```python
from build123d import *

# Parameters (mm, degrees)
SKETCH_1_W                = 80
SKETCH_1_H                = 80
EXTRUDE_1_DEPTH           = 80
HOLE_WIZARD_1_D           = 11
HOLE_WIZARD_1_CBORE_D     = 18
HOLE_WIZARD_1_CBORE_DEPTH = 50
CUT_EXTRUDE_1_DEPTH       = 121


with BuildPart() as part:
    # 草图1 → 凸台-拉伸1 (new body)
    with BuildSketch(Plane(origin=(0, 0, 0), x_dir=(0, 0, -1), z_dir=(1, 0, 0))):
        Rectangle(SKETCH_1_W, SKETCH_1_H)
    extrude(amount=EXTRUDE_1_DEPTH)

    # 打孔尺寸(%根据)内六角圆柱头螺钉的类型1 (through all)
    with Locations(Plane(origin=(80, 0, 0), x_dir=(0, 0, -1), z_dir=(1, 0, 0))):
        with Locations((-25, 0), (25, 0)):
            CounterBoreHole(HOLE_WIZARD_1_D / 2, HOLE_WIZARD_1_CBORE_D / 2, HOLE_WIZARD_1_CBORE_DEPTH)

    # 草图2 → 切除-拉伸1 (cut, through all)
    with BuildSketch(Plane.XY.offset(40)):
        Polygon((20, -40), (80, 20), (80, -40), align=None)
    extrude(amount=-CUT_EXTRUDE_1_DEPTH, mode=Mode.SUBTRACT)


solid = part.part
```
Can you work these out from the model? Positions are in its coordinate system, mm. A direction names the side the tool comes from. Coordinates: 2 decimals unless noted, no trailing zeros. Loops run counter-clockwise (first coordinate to the right, second up) from the corner with the lowest first, then second, coordinate; pieces in that order, holes last.
Item 1: I'm going to push flat-ended pins straight in: pin 1 (9 mm diameter, centred on y = -3, z = 27, fed in from +X); pin 2 (12 mm diameter, centred on x = 56, y = -14.5, fed in from -Z); pin 3 (6 mm diameter, centred on y = -19, z = 17.5, fed in from +X); pin 4 (1.5 mm diameter, centred on x = 35.5, z = -10, fed in from -Y). Where does each tip first touch, or does it pass through?
Answers below:
pin 1: stops at x = 30
pin 2: passes through
pin 3: stops at x = 44
pin 4: stops at y = -25.25
Item 2: Suppose I cut it at D-D (x = 54). Please give me the cut outline in (y, z), then the cut area to 3 significant figures.
Answers below:
outline: (-6, -40) - (40, -40) - (40, 40) - (-6, 40) - (-6, 31.71) arc R9 cw (long way) to (-6, 18.29) - (-6, -18.29) arc R9 cw (long way) to (-6, -31.71) - close
area: 3,230 mm2
Item 3: Please list where these lines run through material, in increasing order: L1, parallel to Y at x = 13.25, z = -25; L2, parallel to Z at x = 47, y = 0; L3, parallel to Z at x = 32, y = -6.
Answers below:
L1: y = -40 to -5.5, 5.5 to 40
L2: z = -40 to -34, -16 to 16, 34 to 40
L3: z = -40 to -31.71, -18.29 to 18.29, 31.71 to 40
Item 4: Suppose I cut it at B-B (x = 33.5). Please give me the cut outline in (y, z).
Answers below:
outline: (-26.5, -40) - (40, -40) - (40, 40) - (-26.5, 40) - close; hole circle Ø18 at (0, -25); hole circle Ø18 at (0, 25)
Item 5: If we mould it in two halves opening along Y, with no side actions, what happens to faces 1 (the face through (31, 8, 40)), 2 (the face through (14.79, -2.11, 30.08)), 3 (the face through (39, 40, 1))? For each: released by +Y, released by -Y, zero draft, split by the parting line, or undercut.
Answers below:
face 1: zero draft
face 2: undercut
face 3: released by +Y
Item 6: Suppose I cut it at A-A (z = -25). Please give me the cut outline in (x, y).
Answers below:
outline: (0, -40) - (20, -40) - (51, -9) - (30, -9) - (30, -5.5) - (0, -5.5) - close; (0, 5.5) - (30, 5.5) - (30, 9) - (69, 9) - (80, 20) - (80, 40) - (0, 40) - close
Item 7: Suppose I cut it at C-C (y = 0). Please give me the cut outline in (x, z).
Answers below:
outline: (0, -40) - (60, -40) - (60, -34) - (30, -34) - (30, -30.5) - (0, -30.5) - close; (0, -19.5) - (30, -19.5) - (30, -16) - (60, -16) - (60, 16) - (30, 16) - (30, 19.5) - (0, 19.5) - close; (0, 30.5) - (30, 30.5) - (30, 34) - (60, 34) - (60, 40) - (0, 40) - close
Item 8: Which directions (+Z, -Z, +X, -X, +Y, -Y) give clear straight access to the entire face, cutting with the end or side of a thin tool? Please do faces 4 (the face through (45.44, 8.923, -23.828)), 5 (the face through (10, -40, 1)).
Answers below:
face 4: +X
face 5: +Z, -Z, +X, -X, -Y
